Job drawing, mm, ordinate dimensions from the low corner. One solid piece. Coordinates: 2 decimals unless noted, no trailing zeros. Write each loop counter-clockwise with the first axis right and the second up, starting at its lowest first coordinate (ties: lowest second). Pieces come first, ordered by that corner, then holes. Notation, with made-up numbers: (7, 35.5) - (35, 35.5) arc R19 cw to (35, 56.5) - close; hole circle Ø3 at (-17.5, 50.25). An arc over 180 degrees is marked (long way). Use a Markdown table: item, result.
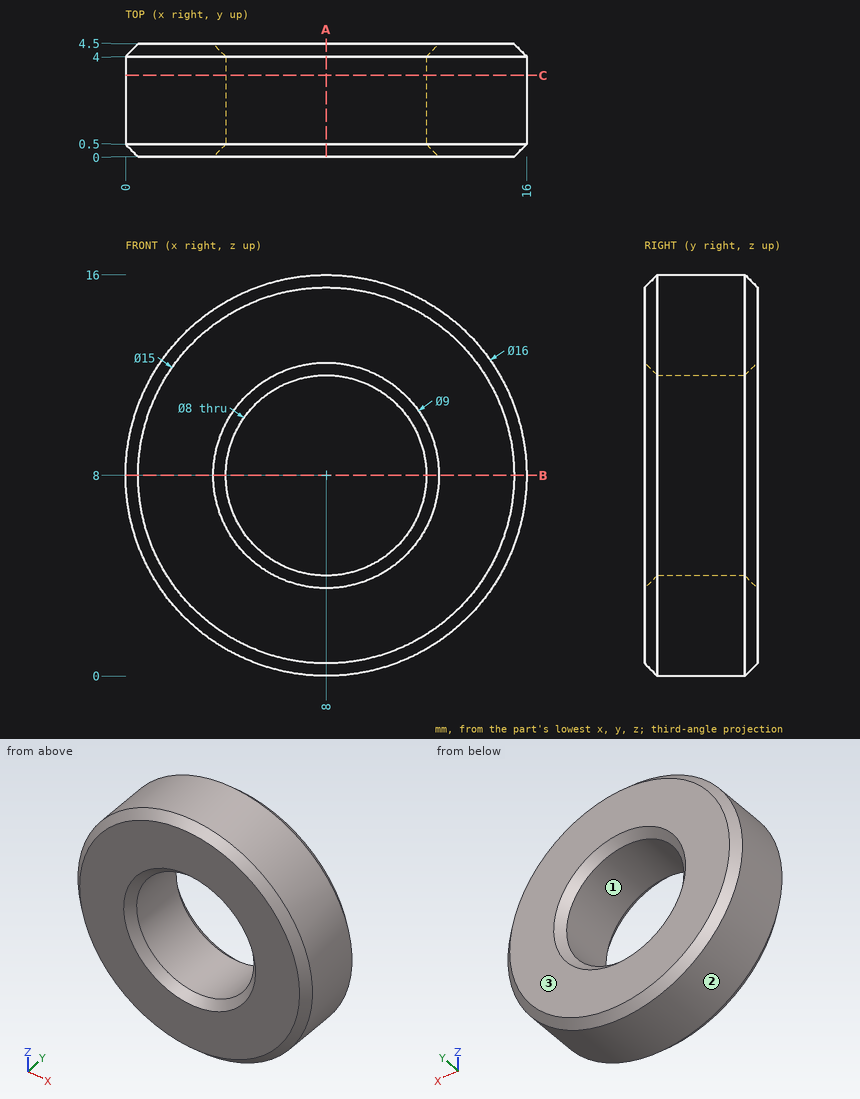
Item 1: Band-saw the part on C-C, the plane y = 3.25. Give the cut face in (x, z).
From the geometry:
| item | result |
|---|---|
| outline | circle Ø16 at (8, 8); hole circle Ø8 at (8, 8) |
Item 2: Two-plate mould, pull along X, no slides. Class the marked faces 1, 2 and 3: pulls with the +X half, pulls with the -X half, needs draft (parallel to the pull), parting line crosses it, or undercut.
From the geometry:
| item | result |
|---|---|
| face 1 | undercut |
| face 2 | parting line crosses it |
| face 3 | needs draft |
Item 3: Drop a flat-ended pin along its axis: P1, Ø1.5, axis at y = 4, z = 5.5, coming from the +X side. Give the stop position or say it passes through.
From the geometry:
| item | result |
|---|---|
| P1 | x = 15.81 |
Item 4: Drill centre lines: probe 1 along X at (y, z) = (3, 8); probe 2 along X at (y, z) = (3.75, 4.5); probe 3 along Z at (x, y) = (7, 3.55). Where is each one in solid material? Low to high.
From the geometry:
| item | result |
|---|---|
| probe 1 | 0 to 4, 12 to 16 |
| probe 2 | 0.81 to 6.06, 9.94 to 15.19 |
| probe 3 | 0.06 to 4.13, 11.87 to 15.94 |
Item 5: Band-saw the part on A-A, the plane x = 8. Give the cut face in (y, z).
From the geometry:
| item | result |
|---|---|
| outline | (0, 0.5) - (0.5, 0) - (4, 0) - (4.5, 0.5) - (4.5, 3.5) - (4, 4) - (0.5, 4) - (0, 3.5) - close; (0, 12.5) - (0.5, 12) - (4, 12) - (4.5, 12.5) - (4.5, 15.5) - (4, 16) - (0.5, 16) - (0, 15.5) - close |
Item 6: Band-saw the part on B-B, the plane z = 8. Give the cut face in (x, y), then the cut area to 3 significant figures.
From the geometry:
| item | result |
|---|---|
| outline | (0, 0.5) - (0.5, 0) - (3.5, 0) - (4, 0.5) - (4, 4) - (3.5, 4.5) - (0.5, 4.5) - (0, 4) - close; (12, 0.5) - (12.5, 0) - (15.5, 0) - (16, 0.5) - (16, 4) - (15.5, 4.5) - (12.5, 4.5) - (12, 4) - close |
| area | 35.0 mm^2 |
